```python
from build123d import *

# Parameters (mm, degrees)
SKETCH1_R                               = 88.9
SKETCH1_R_2                             = 61.975
BOSS_EXTRUDE1_DEPTH                     = 0.381
F_9_16_0_5625_DIAMETER_HOLE1_AT_2_COUNT = 2
F_9_16_0_5625_DIAMETER_HOLE1_AT_2_PITCH = 144.818259586


with BuildPart() as part:
    # Sketch1 → Boss-Extrude1 (new body)
    with BuildSketch(Plane(origin=(0, 0, 0), x_dir=(1, 0, 0), z_dir=(0, 1, 0))):
        with Locations(Location((0, 0, 0), (0, 0, 90))):
            Circle(SKETCH1_R)
        with Locations(Location((0, 0, 0), (0, 0, 90))):
            Circle(SKETCH1_R_2, mode=Mode.SUBTRACT)
    extrude(amount=BOSS_EXTRUDE1_DEPTH)

    # Sketch2 → 9/16 (0.5625) Diameter Hole1 (revolve, cut)
    with BuildSketch(Plane(origin=(-51.6382, 0.381, -51.64), x_dir=(0, 0, 1), z_dir=(1, 0, 0))):
        Polygon((0, 0), (0, 20.172398047), (7.14375, 15.88), (7.14375, 0), align=None)
    f_9_16_0_5625_diameter_hole1 = revolve(axis=Axis((-51.6382, 6.731, -51.64), (0, -1, 0)), mode=Mode.SUBTRACT)

    # 9/16 (0.5625) Diameter Hole1 at 2: 9/16 (0.5625) Diameter Hole1 ×2
    with Locations(*[Vector(0.7932991345710956, 0, 0.6088320647672483) * (i * F_9_16_0_5625_DIAMETER_HOLE1_AT_2_PITCH) for i in range(1, F_9_16_0_5625_DIAMETER_HOLE1_AT_2_COUNT)]):
        add(f_9_16_0_5625_diameter_hole1, mode=Mode.SUBTRACT)

    # Mirror1: 9/16 (0.5625) Diameter Hole1 across plane
    add(f_9_16_0_5625_diameter_hole1.mirror(Plane.XY), mode=Mode.SUBTRACT)

    # Mirror1 copy 1 sketch → Mirror1 copy 1 (revolve, cut)
    with BuildSketch(Plane(origin=(63.246, 0.381, -36.53), x_dir=(0, 0, -1), z_dir=(1, 0, 0))):
        Polygon((0, 0), (0, -20.172398047), (7.14375, -15.88), (7.14375, 0), align=None)
    revolve(axis=Axis((63.246, 6.731, -36.53), (0, 1, 0)), mode=Mode.SUBTRACT)


solid = part.part
```
Part model, mm, in its own coordinate system. Coordinates: 2 decimals unless noted, no trailing zeros. Write each loop counter-clockwise with the first axis right and the second up, starting at its lowest first coordinate (ties: lowest second). Pieces come first, ordered by that corner, then holes.
Item 1: Pin check, flat tip, straight feed: pin 1 (8.5 mm diameter, centred on x = -51.64, z = 51.64, fed in from +Y). Stop position of the tip, or through.
Item 2: Slice it at A-A (z = 0). Write the cut outline in (x, y) (3 decimals).
Item 3: Slice it at B-B (x = 0). Write the cut outline in (y, z) (3 decimals), and give its area (3 significant figures).
Item 4: Probe line 1 (X direction, y = 0.15, z = 0) (3 decimals); line 2 (X direction, y = 0.35, z = -55); line 3 (X direction, y = 0.1, z = -36.53). List the from-to ranges inside material, lowest first.
Item 5: Mould opens along Z. For faces 1 (the face through (-61, 0.381, -19)), 2 (the face through (-74.96, 0.19, -47.79)), 3 (the face through (-58.72, 0.19, 52.57)), 4 (the face through (56.163, 0.193, 35.6)) say: released by +Z, released by -Z, zero draft, split by the parting line, or undercut.
Item 6: Slice it at D-D (y = 0.1). Count the separate pieces of the cut face and the enclosed holes in it, and give its area (3 significant figures).
Item 7: Slice it at C-C (z = -51.64). Write the cut outline in (x, y).
Results found:
1. pin 1: passes through
2. outline: (-88.9, 0) - (-61.975, 0) - (-61.975, 0.381) - (-88.9, 0.381) - close; (61.975, 0) - (88.9, 0) - (88.9, 0.381) - (61.975, 0.381) - close
3. outline: (0, -88.9) - (0.381, -88.9) - (0.381, -61.975) - (0, -61.975) - close; (0, 61.975) - (0.381, 61.975) - (0.381, 88.9) - (0, 88.9) - close
3. area: 20.5 mm2
4. line 1: x = -88.9 to -61.975, 61.975 to 88.9
4. line 2: x = -69.84 to -57.94, -45.33 to -28.56, 28.56 to 69.84
4. line 3: x = -81.05 to -50.06, 50.06 to 56.1, 70.39 to 81.05
5. face 1: zero draft
5. face 2: split by the parting line
5. face 3: undercut
5. face 4: undercut
6. separate pieces: 1
6. enclosed holes: 5
6. area: 12,100 mm2
7. outline: (-72.36, 0) - (-58.78, 0) - (-58.78, 0.38) - (-72.36, 0.38) - close; (-44.49, 0) - (-34.27, 0) - (-34.27, 0.38) - (-44.49, 0.38) - close; (34.27, 0) - (72.36, 0) - (72.36, 0.38) - (34.27, 0.38) - close
